Design review of the part built by this model. Coordinates are the model's own, in mm. A direction names the side the tool comes from. Round coordinates to 2 decimals unless told otherwise and drop trailing zeros. Loops run counter-clockwise (first coordinate to the right, second up) from the corner with the lowest first, then second, coordinate; pieces in that order, holes last. Notation, with made-up numbers: (30, -26.5) - (47, -26.5) arc R22 ccw to (47, -18.5) - close; hole circle Ø3 at (73.25, 27.5). An arc over 180 degrees is marked (long way). One line per question, with ' | ' between items. Start each with the question number.
from build123d import *

# Parameters (mm, degrees)
CLIP_BODY_DEPTH      = 6
ROUNDED_TAB_SKETCH_R = 6
ROUNDED_TAB_DEPTH    = 2
SADDLE_CUT_REACH     = 20.708
PIVOT_HOLE_3_2_REACH = 20.276
PIVOT_HOLE_SKETCH_R  = 1.6
EDGE_FILLETS_R1_R    = 1


with BuildPart() as part:
    # Clip Profile Sketch → Clip Body (new, symmetric)
    with BuildSketch(Plane.XY):
        Polygon((0, -11), (0, 0), (3.4, 0), (3.4, 7), (5, 7), (5, -2), (2, -2), (2, -11), align=None)
    extrude(amount=CLIP_BODY_DEPTH, both=True)

    # Rounded Tab Sketch → Rounded Tab (add)
    with BuildSketch(Plane(origin=(2, 0, 0), x_dir=(0, 0, -1), z_dir=(1, 0, 0))):
        with Locations((0, -11)):
            Circle(ROUNDED_TAB_SKETCH_R)
    extrude(amount=-ROUNDED_TAB_DEPTH)

    # Saddle Cut Sketch → Saddle Cut (cut, up to next)
    with BuildSketch(Plane(origin=(5, 0, 0), x_dir=(0, 0, -1), z_dir=(1, 0, 0)), mode=Mode.PRIVATE) as saddle_cut_sk1:
        with BuildLine():
            Line((-4.5, 7), (4.5, 7))
            ThreePointArc((4.5, 7), (0, 2.5), (-4.5, 7))
        make_face()
    saddle_cut_tool1 = extrude(saddle_cut_sk1.sketch, amount=-SADDLE_CUT_REACH, mode=Mode.PRIVATE) & part.part
    add(saddle_cut_tool1.solids().sort_by_distance((5, 5.090141, 0))[0], mode=Mode.SUBTRACT)

    # Pivot Hole Sketch → Pivot Hole Ø3.2 (cut, up to next)
    with BuildSketch(Plane(origin=(2, 0, 0), x_dir=(0, 0, -1), z_dir=(1, 0, 0)), mode=Mode.PRIVATE) as pivot_hole_3_2_sk1:
        with Locations(Location((0, -11, 0), (0, 0, 90))):
            Circle(PIVOT_HOLE_SKETCH_R)
    pivot_hole_3_2_tool1 = extrude(pivot_hole_3_2_sk1.sketch, amount=-PIVOT_HOLE_3_2_REACH, mode=Mode.PRIVATE) & part.part
    add(pivot_hole_3_2_tool1.solids().sort_by_distance((2, -11, 0))[0], mode=Mode.SUBTRACT)

    # Edge Fillets R1
    edge_fillets_r1_edges = [part.edges().sort_by_distance(p)[0] for p in [
        (0, 0, 0),
        (5, -2, 0),
    ]]
    fillet(edge_fillets_r1_edges, radius=EDGE_FILLETS_R1_R)


solid = part.part
1. Take a section at B-B, the plane z = 0. Give the boundary of the cut face in (x, y).
2. Machinability: for faces 1 (the face through (4, 7, 5)), 2 (the face through (3.4, 2, 0)), 3 (the face through (2, -9, 0)), which of the approach directions +Z, -Z, +X, -X, +Y, -Y give a long, thin tool a straight path to every point of the face, cutting with its end or side? Answer none if there is none.
3. The part is to be moulded in two halves that separate along Y. For faces 4 (the face through (2, 0, 0)), 5 (the face through (0, -9, 0)), 6 (the face through (1.01, -12.6, 0.07)), say which applies: pulls with the +Y half, pulls with the -Y half, needs draft (parallel to the pull), parting line crosses it, or undercut.
4. Take a section at D-D, the plane z = -2.25. Give the boundary of the cut face in (x, y), then the cut area to 3 significant figures.
5. To check wall thickness, follow line 1 along Z through (x, y) = (0.6, -11); line 2 along X through (y, z) = (3, -2.5); line 3 along Y through (x, z) = (2.6, 4.5). State the ranges of each line that lie inside material, in increasing order.
6. Take a section at C-C, the plane y = 4.75. Give the boundary of the cut face in (x, z), then the cut area to 3 significant figures.
7. Clearance check with flat-ended pins moving along their axes: P1, Ø3, axis at y = -11, z = 0, coming from the -X side; P2, Ø2, axis at y = 4, z = 4, coming from the -X side; P3, Ø3, axis at y = -3, z = 4, coming from the +X side; P4, Ø1.2, axis at x = 1.5, z = -1.5, coming from the +Y side. State where each tip first meets the part, or that it passes through.
8. Take a section at A-A, the plane x = 1.3. Give the boundary of the cut face in (y, z).
Answer list:
1) outline: (0, -17) - (2, -17) - (2, -12.6) - (0, -12.6) - close; (0, -9.4) - (2, -9.4) - (2, -2) - (4, -2) arc R1 ccw to (5, -1) - (5, 2.5) - (3.4, 2.5) - (3.4, 0) - (1, 0) arc R1 ccw to (0, -1) - close
2) face 1: +Z, -Z, +X, -X, +Y | face 2: +Z, -Z, -X, +Y | face 3: +Z, -Z, +X, -Y
3) face 4: pulls with the +Y half | face 5: needs draft | face 6: undercut
4) outline: (0, -16.56) - (2, -16.56) - (2, -2) - (4, -2) arc R1 ccw to (5, -1) - (5, 3.1) - (3.4, 3.1) - (3.4, 0) - (1, 0) arc R1 ccw to (0, -1) - close | area: 43.7 mm²
5) line 1: z = -6 to -1.6, 1.6 to 6 | line 2: x = 3.4 to 5 | line 3: y = -2 to 0
6) outline: (3.4, -6) - (5, -6) - (5, -3.9) - (3.4, -3.9) - close; (3.4, 3.9) - (5, 3.9) - (5, 6) - (3.4, 6) - close | area: 6.73 mm²
7) P1: passes through | P2: stops at x = 3.4 | P3: stops at x = 4.87 | P4: stops at y = 0
8) outline: (-11, -6) - (0, -6) - (0, 6) - (-11, 6) arc R6 ccw to start; hole circle Ø3.2 at (-11, 0)
